from build123d import *

# Parameters (mm, degrees)
SKETCH_1_R          = 20
EXTRUDE_1_DEPTH     = 325
SKETCH_2_R          = 27.5
EXTRUDE_2_DEPTH     = 5
CUT_EXTRUDE_1_DEPTH = 10
SKETCH_4_OUTSIDE_W  = 124.808
SKETCH_4_OUTSIDE_H  = 124.808
SKETCH_4_OUTSIDE_R  = 18
CUT_EXTRUDE_2_DEPTH = 25
CHAMFER_1_SIZE      = 1
CHAMFER_2_SIZE      = 1
FILLET_1_R          = 0.5
SKETCH_5_W          = 6
SKETCH_5_H          = 10
CUT_EXTRUDE_3_DEPTH = 25
FILLET_2_R          = 0.5


with BuildPart() as part:
    # 草图1 → 凸台-拉伸1 (new body)
    with BuildSketch(Plane.XY):
        Circle(SKETCH_1_R)
    extrude(amount=EXTRUDE_1_DEPTH)

    # 草图2 → 凸台-拉伸2 (add)
    with BuildSketch(Plane.XY.offset(325)):
        Circle(SKETCH_2_R)
    extrude(amount=EXTRUDE_2_DEPTH)

    # 草图3 → 切除-拉伸1 (cut)
    with BuildSketch(Plane.XY.offset(330)):
        Polygon((9.237604307, 0), (4.618802154, 8), (-4.618802154, 8), (-9.237604307, 0), (-4.618802154, -8), (4.618802154, -8), align=None)
    extrude(amount=-CUT_EXTRUDE_1_DEPTH, mode=Mode.SUBTRACT)

    # 草图4 outside → 切除-拉伸2 (cut)
    with BuildSketch(Plane(origin=(0, 0, 0), x_dir=(-1, 0, 0), z_dir=(0, 0, -1))):
        Rectangle(SKETCH_4_OUTSIDE_W, SKETCH_4_OUTSIDE_H)
        Circle(SKETCH_4_OUTSIDE_R, mode=Mode.SUBTRACT)
    extrude(amount=-CUT_EXTRUDE_2_DEPTH, mode=Mode.SUBTRACT)

    # 倒角1
    chamfer_1_edges = [part.edges().sort_by_distance(p)[0] for p in [
        (-20, 0, 25),
    ]]
    chamfer(chamfer_1_edges, length=CHAMFER_1_SIZE)

    # 倒角2
    chamfer_2_edges = [part.edges().sort_by_distance(p)[0] for p in [
        (18, 0, 0),
    ]]
    chamfer(chamfer_2_edges, length=CHAMFER_2_SIZE)

    # 圆角1
    fillet_1_edges = [part.edges().sort_by_distance(p)[0] for p in [
        (-20, 0, 325),
    ]]
    fillet(fillet_1_edges, radius=FILLET_1_R)

    # 草图5 → 切除-拉伸3 (cut)
    with BuildSketch(Plane(origin=(0, 0, 0), x_dir=(-1, 0, 0), z_dir=(0, 0, -1))):
        with Locations((0, 18)):
            Rectangle(SKETCH_5_W, SKETCH_5_H)
    extrude(amount=-CUT_EXTRUDE_3_DEPTH, mode=Mode.SUBTRACT)

    # 圆角2
    fillet_2_edges = [part.edges().sort_by_distance(p)[0] for p in [
        (-3, 13, 12.5),
        (3, 13, 12.5),
        (3, 17.748239349, 13),
        (-3, 17.748239349, 13),
    ]]
    fillet(fillet_2_edges, radius=FILLET_2_R)


solid = part.part
Part model, mm, in its own coordinate system. A direction names the side the tool comes from. Give positions to 0.01 mm unless a question says otherwise; leave off trailing zeros. Loops run counter-clockwise (first coordinate to the right, second up) from the corner with the lowest first, then second, coordinate; pieces in that order, holes last. Notation, with made-up numbers: (86, 78.25) -> (133, 78.25) arc R8 ccw to (133, 86.25) -> close; hole circle Ø3 at (23.5, -31.5). An arc over 180 degrees is marked (long way). Write each question's results on one line, items separated by ' | '. Start each with the question number.
Q1. Which spindle directions (+Z, -Z, +X, -X, +Y, -Y) get a long thin tool onto all of the face, cutting with end or side? Do faces 1 (the face through (0, 0, 0)), 2 (the face through (-10.3, -18.2, 325)), 3 (the face through (0, 0, 320)). Say none if no direction does.
Q2. Pull direction X, two halves, no side cores. Call faces 4 (the face through (-4.336, -19.524, 173.16)), 5 (the face through (0, -8, 325)), 6 (the face through (6.896, -4.056, 325.07)), 7 (the face through (-6, -6, 330)): +X half, -X half, draft (parallel to the pull), parting line (faces both ways), or undercut.
Q3. Band-saw the part on A-A on z = 248. List the corners of the cut face in (x, y).
Q4. Pin check, flat tips, straight feed: P1, Ø5.5, axis at x = 0.5, z = 18.5, coming from the +Y side; P2, Ø10, axis at x = -2, z = 325.5, coming from the +Y side; P3, Ø5, axis at x = -7, z = 116, coming from the -Y side; P4, Ø2, axis at x = 21.5, z = 208, coming from the +Y side. Stop position of each tip, or through.
Q5. Wall check: L1, parallel to Z at x = 21, y = -8; L2, parallel to Z at x = -5, y = -6.5; L3, parallel to X at y = 1.5, z = 229. Give the ranges that are in metal, low to high.
Results are:
1) face 1: -Z, +X, -X, +Y, -Y | face 2: -Z | face 3: +Z
2) face 4: parting line | face 5: undercut | face 6: undercut | face 7: draft
3) outline: circle Ø40 at (0, 0)
4) P1: stops at y = 17.58 | P2: stops at y = 27.5 | P3: stops at y = -19.49 | P4: passes through
5) L1: z = 325 to 330 | L2: z = 0 to 320 | L3: x = -19.94 to 19.94
